```python
from build123d import *

# Parameters (mm, degrees)
BOSS_EXTRUDE1_DEPTH = 42.5
SKETCH3_W           = 15
SKETCH3_H           = 11
CUT_EXTRUDE2_DEPTH  = 10
SKETCH4_R           = 3
CUT_EXTRUDE3_DEPTH  = 92.332154798


with BuildPart() as part:
    # Sketch1 → Boss-Extrude1 (new, symmetric)
    with BuildSketch(Plane(origin=(0, 0, 0), x_dir=(0, 0, -1), z_dir=(1, 0, 0))):
        with BuildLine():
            Line((5.099019514, -1.25), (33, -1.25))
            Line((33, -1.25), (33, -5.25))
            Line((33, -5.25), (0, -5.25))
            ThreePointArc((0, -5.25), (-3.240370349, 4.13067791), (5.099019514, -1.25))
        make_face()
    extrude(amount=BOSS_EXTRUDE1_DEPTH, both=True)

    # Sketch3 → Cut-Extrude2 (cut, symmetric)
    with BuildSketch(Plane(origin=(0, 0, 0), x_dir=(1, 0, 0), z_dir=(0, 1, 0))):
        with Locations((14, 0)):
            Rectangle(SKETCH3_W, SKETCH3_H)
        with Locations((-14, 0)):
            Rectangle(SKETCH3_W, SKETCH3_H)
    extrude(amount=CUT_EXTRUDE2_DEPTH, both=True, mode=Mode.SUBTRACT)

    # Sketch4 → Cut-Extrude3 (cut, through all)
    with BuildSketch(Plane(origin=(42.5, 0, 0), x_dir=(0, 0, -1), z_dir=(1, 0, 0))):
        Circle(SKETCH4_R)
    extrude(amount=-CUT_EXTRUDE3_DEPTH, mode=Mode.SUBTRACT)


solid = part.part
```
Read the model definition and answer for the solid it produces. Units are mm, in the model's axes. A direction names the side the tool comes from. Give positions to 0.01 mm unless a question says otherwise; leave off trailing zeros. Order: outer loops, then holes, each group sorted by start corner. A loop starts at its lowest first (then second) coordinate and runs counter-clockwise, first axis right, second up.
(1) Find section B-B (x = -28). Give the vertices of the cut face in (y, z), plus the area to 3 significant figures.
(2) Find section A-A (y = 0). Give the vertices of the cut face in (x, z), plus the area to 4 significant figures.
(3) Straight lines are drawn through the part: L1, parallel to Y at x = 27, z = 0; L2, parallel to X at y = 3, z = -3; L3, parallel to Y at x = 6, z = -8. For each, find the intervals that lie inside material, in ascending order.
(4) Find section C-C (z = -1.5). Give the vertices of the cut face in (x, y), plus the area to 3 significant figures.
(5) For a pull along Z with two mould halves and no side action, classify faces 3 (the flat face through (21.5, -2.4, -2.4)), 4 (the cylindrical face through (0, 0, 3)), 5 (the flat face through (1, -3, -33)) as released by +Z, released by -Z, zero draft, split by the parting line, or undercut.
(6) Given pin 1 (14 mm diameter, centred on x = 15, z = -16, fed in from +Y); pin 2 (4.5 mm diameter, centred on x = -13.5, y = -2.5, fed in from +Z); pin 3 (12 mm diameter, centred on x = -8.5, z = -6, fed in from +Y), each flat-ended and moving along its own axis, determine where each tip first touches the part or whether it passes through.
(7) For faces 1 (the flat face through (-14, -3, -5.5)), 2 (the cylindrical face through (32, 0, 3)), determine the directions among +Z, -Z, +X, -X, +Y, -Y from which every point of the face is accessible in a straight line to the end or side of a thin tool.
(8) Find section D-D (x = 8). Give the vertices of the cut face in (y, z).
Result sheet:
1. outline: (-5.25, -33) - (-1.25, -33) - (-1.25, -5.1) arc R5.25 ccw (long way) to (-5.25, 0) - close; hole circle Ø6 at (0, 0)
1. area: 175 mm2
2. outline: (-42.5, -5.25) - (-21.5, -5.25) - (-21.5, -3) - (-42.5, -3) - close; (-42.5, 3) - (-21.5, 3) - (-21.5, 5.25) - (-42.5, 5.25) - close; (-6.5, -5.25) - (6.5, -5.25) - (6.5, -3) - (-6.5, -3) - close; (-6.5, 3) - (6.5, 3) - (6.5, 5.25) - (-6.5, 5.25) - close; (21.5, -5.25) - (42.5, -5.25) - (42.5, -3) - (21.5, -3) - close; (21.5, 3) - (42.5, 3) - (42.5, 5.25) - (21.5, 5.25) - close
2. area: 247.5 mm2
3. L1: y = -5.25 to -3, 3 to 5.25
3. L2: x = -42.5 to -21.5, -6.5 to 6.5, 21.5 to 42.5
3. L3: y = -5.25 to -1.25
4. outline: (-42.5, -5.25) - (-21.5, -5.25) - (-21.5, -2.6) - (-42.5, -2.6) - close; (-42.5, 2.6) - (-21.5, 2.6) - (-21.5, 5.03) - (-42.5, 5.03) - close; (-6.5, -5.25) - (6.5, -5.25) - (6.5, -2.6) - (-6.5, -2.6) - close; (-6.5, 2.6) - (6.5, 2.6) - (6.5, 5.03) - (-6.5, 5.03) - close; (21.5, -5.25) - (42.5, -5.25) - (42.5, -2.6) - (21.5, -2.6) - close; (21.5, 2.6) - (42.5, 2.6) - (42.5, 5.03) - (21.5, 5.03) - close
4. area: 280 mm2
5. face 3: zero draft
5. face 4: undercut
5. face 5: released by -Z
6. pin 1: stops at y = -1.25
6. pin 2: stops at z = -5.5
6. pin 3: stops at y = 5.24
7. face 1: +Z, +Y, -Y
7. face 2: +X, -X
8. outline: (-5.25, -33) - (-1.25, -33) - (-1.25, -5.5) - (-5.25, -5.5) - close
